Can you work these out from the model? Positions are in its coordinate system, mm. Round coordinates to 2 decimals unless told otherwise and drop trailing zeros. Order: outer loops, then holes, each group sorted by start corner. A loop starts at its lowest first (then second) coordinate and runs counter-clockwise, first axis right, second up. Notation, with made-up numbers: M -19,46 L 26,46 A9 ccw 26,60 Z; hole C 70.5,32 d9. An arc over 180 degrees is marked long. Answer as a JSON object with one key per item and string values. Group by question number.
from build123d import *

# Parameters (mm, degrees)
BOSS_EXTRUDE1_DEPTH    = 2455
CUT_EXTRUDE1_DEPTH     = 2471.34516819
CUT_EXTRUDE2_DEPTH     = 10
M10_TAPPED_HOLE1_D     = 8.5
M10_TAPPED_HOLE1_DEPTH = 27.5
M10_TAPPED_HOLE1_TIP   = 2.553657631


with BuildPart() as part:
    # Sketch1 → Boss-Extrude1 (new body)
    with BuildSketch(Plane.XY):
        with BuildLine():
            Line((-147.5, 0), (-147.5, 166.076644929))
            ThreePointArc((-147.5, 166.076644929), (-141.615705819, 183.921328531), (-126.271151142, 194.765787607))
            Line((-126.271151142, 194.765787607), (-8.771151142, 230.689142679))
            ThreePointArc((-8.771151142, 230.689142679), (0, 232), (8.771151142, 230.689142679))
            Line((8.771151142, 230.689142679), (126.271151142, 194.765787607))
            ThreePointArc((126.271151142, 194.765787607), (141.615705819, 183.921328531), (147.5, 166.076644929))
            Line((147.5, 166.076644929), (147.5, 0))
            Line((147.5, 0), (137.5, 0))
            Line((137.5, 0), (137.5, 166.076644929))
            ThreePointArc((137.5, 166.076644929), (133.577137212, 177.973100664), (123.347434094, 185.202740048))
            Line((123.347434094, 185.202740048), (5.847434094, 221.126095119))
            ThreePointArc((5.847434094, 221.126095119), (0, 222), (-5.847434094, 221.126095119))
            Line((-5.847434094, 221.126095119), (-123.347434094, 185.202740048))
            ThreePointArc((-123.347434094, 185.202740048), (-133.577137212, 177.973100664), (-137.5, 166.076644929))
            Line((-137.5, 166.076644929), (-137.5, 0))
            Line((-137.5, 0), (-147.5, 0))
        make_face()
    extrude(amount=BOSS_EXTRUDE1_DEPTH)

    # Sketch2 → Cut-Extrude1 (cut, through all)
    with BuildSketch(Plane(origin=(0, 0, 0), x_dir=(1, 0, 0), z_dir=(0, 1, 0))):
        with BuildLine():
            Line((-70, -1975), (-70, -2455))
            Line((-70, -2455), (70, -2455))
            Line((70, -2455), (70, -1975))
            ThreePointArc((70, -1975), (0, -1905), (-70, -1975))
        make_face()
    extrude(amount=CUT_EXTRUDE1_DEPTH, mode=Mode.SUBTRACT)

    # Sketch3 → Cut-Extrude2 (cut)
    with BuildSketch(Plane.ZY.offset(147.5)):
        with BuildLine():
            Line((1545, 137), (1585, 137))
            ThreePointArc((1585, 137), (1625, 97), (1585, 57))
            Line((1585, 57), (1545, 57))
            ThreePointArc((1545, 57), (1505, 97), (1545, 137))
        make_face()
    extrude(amount=-CUT_EXTRUDE2_DEPTH, mode=Mode.SUBTRACT)

    # M10 Tapped Hole1
    with Locations(Plane.ZY.offset(147.5)):
        with Locations((1565, 147), (1565, 47), (1495, 97), (1635, 97)):
            Hole(M10_TAPPED_HOLE1_D / 2, depth=M10_TAPPED_HOLE1_DEPTH)
            with Locations((0, 0, -(M10_TAPPED_HOLE1_DEPTH + M10_TAPPED_HOLE1_TIP / 2))):  # 118° drill point
                Cone(0, M10_TAPPED_HOLE1_D / 2, M10_TAPPED_HOLE1_TIP, mode=Mode.SUBTRACT)


solid = part.part
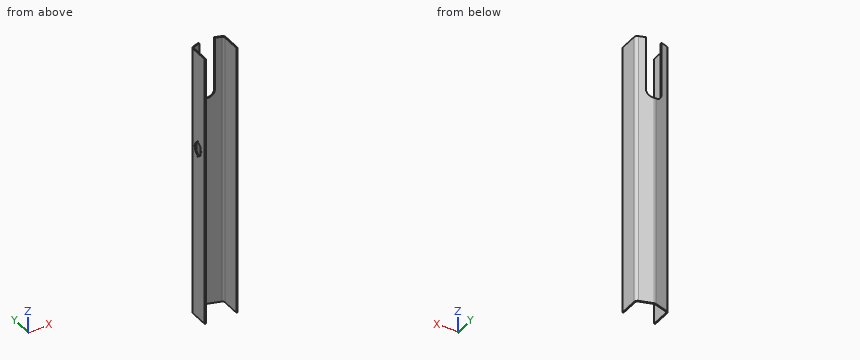
Item 1: I'm going to push flat-ended pins straight in: pin 1 Ø8 at (x, z) = (-144.5, 1568) entering from -Y; pin 2 Ø5 at (x, z) = (-62.5, 1058.5) entering from -Y; pin 3 Ø3 at (x, z) = (-72, 1437.5) entering from +Y; pin 4 Ø7 at (y, z) = (47, 1565) entering from -X. Where does each tip first touch, or does it pass through?
Item 2: Suppose I cut it at A-A, the plane z = 618. Write out the boundary of the cut face in (x, y).
Item 3: I need wall thicknesses on line 1 (Y direction, x = -142, z = 1565); line 2 (X direction, y = 81, z = 1378); line 3 (Y direction, x = -141.5, z = 1565). Which ranges of each line are inside material? Lowest first, please.
Computed:
{
 "1": {"pin 1": "stops at y = 0", "pin 2": "stops at y = 203.04", "pin 3": "stops at y = 211.82", "pin 4": "stops at x = 137.5"},
 "2": {"outline": "M -147.5,0 L -137.5,0 L -137.5,166.08 A20 cw -123.35,185.2 L -5.85,221.13 A20 cw 5.85,221.13 L 123.35,185.2 A20 cw 137.5,166.08 L 137.5,0 L 147.5,0 L 147.5,166.08 A30 ccw 126.27,194.77 L 8.77,230.69 A30 ccw -8.77,230.69 L -126.27,194.77 A30 ccw -147.5,166.08 Z"},
 "3": {"line 1": "y = 0 to 42.75, 51.25 to 57, 137 to 142.75, 151.25 to 183.39", "line 2": "x = -147.5 to -137.5, 137.5 to 147.5", "line 3": "y = 0 to 42.75, 51.25 to 57, 137 to 142.75, 151.25 to 184.08"}
}
